Could you check a few things on this model? Use its own coordinates, in mm. Give positions to 0.01 mm unless a question says otherwise; leave off trailing zeros. Order: outer loops, then holes, each group sorted by start corner. A loop starts at its lowest first (then second) coordinate and runs counter-clockwise, first axis right, second up. Notation, with made-up numbers: (79, -35) -> (97, -35) arc R8 cw to (97, -29) -> close; hole circle Ø2 at (47, 47.25). An arc over 180 degrees is marked (long way). Use one line per item in the form item = value. Start each with the question number.
from build123d import *

# Parameters (mm, degrees)
SKETCH1_R           = 1.5
BOSS_EXTRUDE1_DEPTH = 0.5
SKETCH2_R           = 0.5
CUT_EXTRUDE1_DEPTH  = 16.358222553


with BuildPart() as part:
    # Sketch1 → Boss-Extrude1 (new body)
    with BuildSketch(Plane(origin=(0, 0, 0), x_dir=(1, 0, 0), z_dir=(0, 1, 0))):
        with BuildLine():
            Line((12.75, 2), (3.75, 2))
            ThreePointArc((3.75, 2), (-4.25, 0), (3.75, -2))
            Line((3.75, -2), (12.75, -2))
            ThreePointArc((12.75, -2), (14.75, 0), (12.75, 2))
        make_face()
        with Locations(Location((0, 0, 0), (0, 0, 270))):
            Circle(SKETCH1_R, mode=Mode.SUBTRACT)
    extrude(amount=BOSS_EXTRUDE1_DEPTH)

    # Sketch2 → Cut-Extrude1 (cut, through all)
    with BuildSketch(Plane(origin=(0, 0.5, 0), x_dir=(1, 0, 0), z_dir=(0, 1, 0))):
        with Locations((12, 2.32)):
            Circle(SKETCH2_R)
        with Locations((12, -2.32)):
            Circle(SKETCH2_R)
    extrude(amount=-CUT_EXTRUDE1_DEPTH, mode=Mode.SUBTRACT)


solid = part.part
(1) Please list where these lines run through material, in increasing order: probe 1 along X at (y, z) = (0.3, 0); probe 2 along Z at (x, y) = (6.75, 0.15); probe 3 along X at (y, z) = (0.1, -0.5).
(2) Imagine slicing it at A-A (z = 0). Write out the boundary of the cut face in (x, y).
(3) We'd pull the mould along X, two halves only. Please class faces 1 (the cylindrical face through (-4.247, 0.246, -0.158)), 2 (the cylindrical face through (14.75, 0.25, 0.04)), 3 (the flat face through (5, 0.5, 0)), 4 (the cylindrical face through (0.45, 0.25, 1.43)): pulls with the +X half, pulls with the -X half, needs draft (parallel to the pull), parting line crosses it, or undercut.
(4) Imagine slicing it at B-B (y = 0.2). Write out the boundary of the cut face in (x, z).
(5) Imagine slicing it at D-D (x = 4). Write out the boundary of the cut face in (y, z), plus the area to 3 significant figures.
(6) Imagine slicing it at C-C (x = 0). Write out the boundary of the cut face in (y, z), plus the area to 3 significant figures.
Calculated:
q1.probe_1 = -4.25 to -1.5, 1.5 to 14.75
q1.probe_2 = -2 to 2
q1.probe_3 = -4.22 to -1.41, 1.41 to 14.69
q2.outline = (-4.25, 0) -> (-1.5, 0) -> (-1.5, 0.5) -> (-4.25, 0.5) -> close; (1.5, 0) -> (14.75, 0) -> (14.75, 0.5) -> (1.5, 0.5) -> close
q3.face_1 = parting line crosses it
q3.face_2 = pulls with the +X half
q3.face_3 = needs draft
q3.face_4 = undercut
q4.outline = (3.75, -2) -> (11.62, -2) arc R0.5 cw to (12.38, -2) -> (12.75, -2) arc R2 ccw to (12.75, 2) -> (12.38, 2) arc R0.5 cw to (11.62, 2) -> (3.75, 2) arc R4.25 ccw (long way) to start; hole circle Ø3 at (0, 0)
q5.outline = (0, -2) -> (0.5, -2) -> (0.5, 2) -> (0, 2) -> close
q5.area = 2.00 mm2
q6.outline = (0, -4.25) -> (0.5, -4.25) -> (0.5, -1.5) -> (0, -1.5) -> close; (0, 1.5) -> (0.5, 1.5) -> (0.5, 4.25) -> (0, 4.25) -> close
q6.area = 2.75 mm2
